from build123d import *

# Parameters (mm, degrees)
SKETCH2_W          = 12
SKETCH2_H          = 12
CUT_EXTRUDE1_DEPTH = 90.412028951
SKETCH3_R          = 1.5
CUT_EXTRUDE2_DEPTH = 10


with BuildPart() as part:
    # Sketch1 → Revolve1 (revolve)
    with BuildSketch(Plane.XY, mode=Mode.PRIVATE) as revolve1_sk:
        Polygon((0, 25), (0, 35), (5, 35), (5, 32), (10, 32), (10, 35), (20, 35), (20, 40), (50, 50.919107028), (50, 37.5), (53, 37.5), (53, 25), align=None)
    revolve(revolve1_sk.sketch.rotate(Axis((0, 0, 0), (1, 0, 0)), 90), axis=Axis((0, 0, 0), (1, 0, 0)))

    # Sketch2 → Cut-Extrude1 (cut, through all)
    with BuildSketch(Plane(origin=(53, 0, 0), x_dir=(0, 0, -1), z_dir=(1, 0, 0))):
        with Locations((0, 24)):
            Rectangle(SKETCH2_W, SKETCH2_H)
    extrude(amount=-CUT_EXTRUDE1_DEPTH, mode=Mode.SUBTRACT)

    # Sketch3 → Cut-Extrude2 (cut)
    with BuildSketch(Plane(origin=(53, 0, 0), x_dir=(0, 0, -1), z_dir=(1, 0, 0))):
        with Locations((0, -32.5)):
            Circle(SKETCH3_R)
    extrude(amount=-CUT_EXTRUDE2_DEPTH, mode=Mode.SUBTRACT)


solid = part.part
The model under review builds one solid part; all positions refer to its coordinate system, in mm. A direction names the side the tool comes from. Round coordinates to 2 decimals unless told otherwise and drop trailing zeros. Write each loop counter-clockwise with the first axis right and the second up, starting at its lowest first coordinate (ties: lowest second). Pieces come first, ordered by that corner, then holes. Notation, with made-up numbers: (79, -0.75) - (110, -0.75) arc R11 cw to (110, 11.25) - close; hole circle Ø3 at (-29, 18). An arc over 180 degrees is marked (long way). One line per item, written item: value. Start each with the question number.
1. Consider section D-D on x = 39.5. Write out the cut boundary in (y, z).
2. To check wall thickness, follow L1, parallel to Y at x = 49, z = 0; L2, parallel to Y at x = 48, z = 0; L3, parallel to X at y = -26.5, z = -18. State the ranges of each line that lie inside material, in increasing order. Write a range as from..to.
3. Machinability: for faces 4 (the face through (15.07, 34.168, -7.587)), 5 (the face through (27, 27, -6)), 6 (the face through (5, 28.4, 15.4)), which of the approach directions +Z, -Z, +X, -X, +Y, -Y give a long, thin tool a straight path to every point of the face, cutting with its end or side? Answer none if there is none.
4. Consider section A-A on z = 0. Write out the cut boundary in (x, y).
5. Consider section C-C on x = 46.5. Write out the cut boundary in (y, z).
6. The part is to be moulded in two halves that separate along X. For faces 1 (the face through (27, 30, 0)), 2 (the face through (7.54, 31.24, -6.94)), 3 (the face through (43, -32, 0)), say which applies: released by +X, released by -X, zero draft, split by the parting line, or undercut.
7. Clearance check with flat-ended pins moving along their axes: P1, Ø24, axis at y = -1.5, z = 4.5, coming from the -X side; P2, Ø21, axis at y = -8.5, z = -16, coming from the +X side; P3, Ø13, axis at x = 24.5, z = 0.5, coming from the -Y side; P4, Ø0.9, axis at y = -33, z = 0, coming from the +X side. State where each tip first meets the part, or that it passes through.
8. Consider section B-B on y = 0. Write out the cut boundary in (x, z).
Checks:
1. outline: circle Ø94.19 at (0, 0); hole (24.27, -6) - (30, -6) - (30, 6) - (24.27, 6) arc R25 ccw (long way) to start
2. L1: y = -50.56..-34, -31..-25, 30..50.56
2. L2: y = -50.19..-34, -31..-25, 30..50.19
2. L3: x = 0..5, 10..53
3. face 4: -X
3. face 5: +X, -X
3. face 6: none
4. outline: (0, -35) - (5, -35) - (5, -32) - (10, -32) - (10, -35) - (20, -35) - (20, -40) - (50, -50.92) - (50, -37.5) - (53, -37.5) - (53, -34) - (43, -34) - (43, -31) - (53, -31) - (53, -25) - (0, -25) - close; (0, 30) - (53, 30) - (53, 37.5) - (50, 37.5) - (50, 50.92) - (20, 40) - (20, 35) - (10, 35) - (10, 32) - (5, 32) - (5, 35) - (0, 35) - close
5. outline: circle Ø99.29 at (0, 0); hole circle Ø3 at (-32.5, 0); hole (24.27, -6) - (30, -6) - (30, 6) - (24.27, 6) arc R25 ccw (long way) to start
6. face 1: zero draft
6. face 2: undercut
6. face 3: released by +X
7. P1: passes through
7. P2: stops at x = 53
7. P3: stops at y = -44
7. P4: stops at x = 43
8. outline: (0, -35) - (5, -35) - (5, -32) - (10, -32) - (10, -35) - (20, -35) - (20, -40) - (50, -50.92) - (50, -37.5) - (53, -37.5) - (53, -25) - (0, -25) - close; (0, 25) - (53, 25) - (53, 37.5) - (50, 37.5) - (50, 50.92) - (20, 40) - (20, 35) - (10, 35) - (10, 32) - (5, 32) - (5, 35) - (0, 35) - close
